from build123d import *

# Parameters (mm, degrees)
SKETCH1_W             = 45
SKETCH1_H             = 50
BOSS_EXTRUDE1_DEPTH   = 10
CUT_EXTRUDE1_DEPTH    = 59.854546763
CHAMFER1_SIZE         = 5
M6_TAPPED_HOLE1_D     = 5
M6_TAPPED_HOLE1_DEPTH = 19
M6_TAPPED_HOLE1_TIP   = 1.502151548


with BuildPart() as part:
    # Sketch1 → Boss-Extrude1 (new body)
    with BuildSketch(Plane.XY):
        with Locations((-10.287049861, 22.842105263)):
            Rectangle(SKETCH1_W, SKETCH1_H)
    extrude(amount=BOSS_EXTRUDE1_DEPTH)

    # Sketch2 → Cut-Extrude1 (cut, through all)
    with BuildSketch(Plane.XY.offset(10)):
        with BuildLine():
            Line((-13.537049861, 40.342105263), (-13.537049861, 10.342105263))
            ThreePointArc((-13.537049861, 10.342105263), (-17.787049861, 6.092105263), (-22.037049861, 10.342105263))
            Line((-22.037049861, 10.342105263), (-22.037049861, 40.342105263))
            ThreePointArc((-22.037049861, 40.342105263), (-17.787049861, 44.592105263), (-13.537049861, 40.342105263))
        make_face()
    extrude(amount=-CUT_EXTRUDE1_DEPTH, mode=Mode.SUBTRACT)

    # Chamfer1
    chamfer1_edges = [part.edges().sort_by_distance(p)[0] for p in [
        (-32.787049861, 47.842105263, 5),
        (-32.787049861, -2.157894737, 5),
    ]]
    chamfer(chamfer1_edges, length=CHAMFER1_SIZE)

    # M6 Tapped Hole1
    with Locations(Plane(origin=(12.212950139, 0, 0), x_dir=(0, 0, -1), z_dir=(1, 0, 0))):
        with Locations((-5, 32.842105263), (-5, 2.842105263)):
            Hole(M6_TAPPED_HOLE1_D / 2, depth=M6_TAPPED_HOLE1_DEPTH)
            with Locations((0, 0, -(M6_TAPPED_HOLE1_DEPTH + M6_TAPPED_HOLE1_TIP / 2))):  # 118° drill point
                Cone(0, M6_TAPPED_HOLE1_D / 2, M6_TAPPED_HOLE1_TIP, mode=Mode.SUBTRACT)


solid = part.part
Model file for the job. Use its own axes, mm. A direction names the side the tool comes from. Round coordinates to 2 decimals unless told otherwise and drop trailing zeros. Order: outer loops, then holes, each group sorted by start corner. A loop starts at its lowest first (then second) coordinate and runs counter-clockwise, first axis right, second up.
(1) Band-saw the part on C-C (x = -30). List the corners of the cut face in (y, z).
(2) 3-axis set-ups, long thin cutter, end or side, ignore diameter. For faces 1 (the face through (-30.25, 45.38, 4.93)), 2 (the face through (-13.537, 26, 5)), 3 (the face through (2.58, 3.593, 7.385)): which of +Z, -Z, +X, -X, +Y, -Y reach the whole face in a straight line?
(3) Band-saw the part on A-A (y = 36.5). List the corners of the cut face in (x, z), then the cut area to 3 significant figures.
(4) Band-saw the part on B-B (z = 8.5). List the corners of the cut face in (x, y).
(5) Drill centre lines: line 1 (Y direction, x = 7.25, z = 5); line 2 (Y direction, x = 2, z = 5.25); line 3 (X direction, y = 38.5, z = 3). Where is each one in solid material? Low to high.
(6) Pull direction Z, two halves, no side cores. Call faces 4 (the face through (-11, 23, 10)), 5 (the face through (12.213, 22, 5)), 6 (the face through (2.58, 34.95, 6.344)), 7 (the face through (-11, 23, 0)): released by +Z, released by -Z, zero draft, split by the parting line, or undercut.
(7) Pin check, flat tip, straight feed: pin 1 (4.5 mm diameter, centred on y = 2.84, z = 5, fed in from +X). Stop position of the tip, or through.
Verdict:
1. outline: (0.06, 0) - (45.63, 0) - (45.63, 10) - (0.06, 10) - close
2. face 1: +Z, -Z, -X, +Y
2. face 2: +Z, -Z
2. face 3: +X
3. outline: (-32.79, 0) - (-22.04, 0) - (-22.04, 10) - (-32.79, 10) - close; (-13.54, 0) - (12.21, 0) - (12.21, 10) - (-13.54, 10) - close
3. area: 365 mm2
4. outline: (-32.79, 2.84) - (-27.79, -2.16) - (12.21, -2.16) - (12.21, 47.84) - (-27.79, 47.84) - (-32.79, 42.84) - close; hole (-22.04, 10.34) arc R4.25 ccw to (-13.54, 10.34) - (-13.54, 40.34) arc R4.25 ccw to (-22.04, 40.34) - close
5. line 1: y = -2.16 to 0.34, 5.34 to 30.34, 35.34 to 47.84
5. line 2: y = -2.16 to 0.35, 5.33 to 30.35, 35.33 to 47.84
5. line 3: x = -32.79 to -22.04, -13.54 to 12.21
6. face 4: released by +Z
6. face 5: zero draft
6. face 6: undercut
6. face 7: released by -Z
7. pin 1: stops at x = -6.94
